```python
from build123d import *

# Parameters (mm, degrees)
MAIN_BLOCK_PROFILE_W            = 44
MAIN_BLOCK_PROFILE_H            = 46
MAIN_BLOCK_PROFILE_R            = 11
MAIN_BLOCK_44MM_DEPTH           = 44
TOP_POCKET_PROFILE_28X28_W      = 28
TOP_POCKET_PROFILE_28X28_H      = 28
TOP_SQUARE_POCKET_28X28X5_DEPTH = 5
SIDE_BOSS_PROFILE_W             = 26
SIDE_BOSS_PROFILE_H             = 30
SIDE_BOSS_PROFILE_W_2           = 14
SIDE_BOSS_PROFILE_H_2           = 16
SIDE_SQUARE_BOSS_23MM_DEPTH     = 23
SIDE_OPENING_PROFILE_W          = 14
SIDE_OPENING_PROFILE_H          = 16
SIDE_OPENING_CUT_DEPTH          = 103.786185842


with BuildPart() as part:
    # Main Block Profile → Main Block 44mm (new body)
    with BuildSketch(Plane.XY):
        Rectangle(MAIN_BLOCK_PROFILE_W, MAIN_BLOCK_PROFILE_H)
        with Locations((0, -1)):
            Circle(MAIN_BLOCK_PROFILE_R, mode=Mode.SUBTRACT)
    extrude(amount=-MAIN_BLOCK_44MM_DEPTH)

    # Top Pocket Profile 28x28 → Top Square Pocket 28x28x5 (cut)
    with BuildSketch(Plane(origin=(0, 23, 0), x_dir=(1, 0, 0), z_dir=(0, 1, 0))):
        with Locations((0, 22)):
            Rectangle(TOP_POCKET_PROFILE_28X28_W, TOP_POCKET_PROFILE_28X28_H)
    extrude(amount=-TOP_SQUARE_POCKET_28X28X5_DEPTH, mode=Mode.SUBTRACT)

    # Side Boss Profile → Side Square Boss 23mm (add)
    with BuildSketch(Plane.ZY.offset(22)):
        with Locations((-16, 0)):
            Rectangle(SIDE_BOSS_PROFILE_W, SIDE_BOSS_PROFILE_H)
        with Locations((-16, 0)):
            Rectangle(SIDE_BOSS_PROFILE_W_2, SIDE_BOSS_PROFILE_H_2, mode=Mode.SUBTRACT)
    side_square_boss_23mm = extrude(amount=SIDE_SQUARE_BOSS_23MM_DEPTH)

    # Side Boss Mirror: Side Square Boss 23mm across plane
    add(side_square_boss_23mm.mirror(Plane(origin=(0, 0, 0), x_dir=(0, 0, 1), z_dir=(1, 0, 0))))

    # Side Opening Profile → Side Opening Cut (cut, through all)
    with BuildSketch(Plane(origin=(45, 0, 0), x_dir=(0, 0, -1), z_dir=(1, 0, 0))):
        with Locations((16, 0)):
            Rectangle(SIDE_OPENING_PROFILE_W, SIDE_OPENING_PROFILE_H)
    extrude(amount=-SIDE_OPENING_CUT_DEPTH, mode=Mode.SUBTRACT)


solid = part.part
```
Work out the finished part from the listing and answer in its coordinate system (mm). A direction names the side the tool comes from. Round coordinates to 2 decimals unless told otherwise and drop trailing zeros. Write each loop counter-clockwise with the first axis right and the second up, starting at its lowest first coordinate (ties: lowest second). Pieces come first, ordered by that corner, then holes. Notation, with made-up numbers: (22, -33.75) - (27, -33.75) arc R24 cw to (27, -14.75) - close; hole circle Ø2 at (67.5, -2). An arc over 180 degrees is marked (long way). Return JSON: item names as keys, results as strings. Group by question number.
Q1. The part is cut by section D-D on y = -1. Write down the section's boundary in (x, z).
Q2. The mould has two halves that part along Y. Classify faces 4 (the flat face through (0, 18, -22)), 5 (the cylindrical face through (5.914, 8.275, -21.692)), 6 (the flat face through (45, 0, -8)): released by +Y, released by -Y, zero draft, split by the parting line, or undercut.
Q3. The part is cut by section C-C on x = -21. Write down the section's boundary in (y, z).
Q4. For faces 1 (the flat face through (26, 0, -9)), 2 (the flat face through (-33, 0, -29)), 3 (the flat face through (33, 0, -3)), determine the directions among +Z, -Z, +X, -X, +Y, -Y from which every point of the face is accessible in a straight line to the end or side of a thin tool.
Q5. Each of these flat-tipped pins is pushed along its axis until it touches: pin 1 Ø8 at (x, y) = (32, -2) entering from +Z; pin 2 Ø18.5 at (x, y) = (-36.5, 1.5) entering from -Z; pin 3 Ø12 at (x, z) = (-29.5, -10) entering from +Y; pin 4 Ø17.5 at (x, y) = (0, -1) entering from -Z. Where does it stop, or does it pass through?
Q6. The part is cut by section B-B on z = -22. Write down the section's boundary in (x, y).
Q7. Find the intervals of material crossed by L1, parallel to Y at x = 0, z = -21; L2, parallel to X at y = -1, z = -25.5; L3, parallel to X at y = -1, z = -34, in increasing order.
Q8. The part is cut by section A-A on x = 0. Write down the section's boundary in (y, z), then the cut area to 3 significant figures.
Solved:
{
 "1": {"outline": "(-45, -29) - (-22, -29) - (-22, -44) - (-11, -44) - (-11, -23) - (-45, -23) - close; (-45, -9) - (-11, -9) - (-11, 0) - (-22, 0) - (-22, -3) - (-45, -3) - close; (11, -44) - (22, -44) - (22, -29) - (45, -29) - (45, -23) - (11, -23) - close; (11, -9) - (45, -9) - (45, -3) - (22, -3) - (22, 0) - (11, 0) - close"},
 "2": {"face 4": "released by +Y", "face 5": "undercut", "face 6": "zero draft"},
 "3": {"outline": "(-23, -44) - (23, -44) - (23, 0) - (-23, 0) - close; hole (-8, -23) - (8, -23) - (8, -9) - (-8, -9) - close"},
 "4": {"face 1": "+X, -X", "face 2": "-Z, -X, +Y, -Y", "face 3": "+Z, +X, +Y, -Y"},
 "5": {"pin 1": "z = -3", "pin 2": "z = -29", "pin 3": "y = 15", "pin 4": "through"},
 "6": {"outline": "(-45, -15) - (-22, -15) - (-22, -23) - (22, -23) - (22, -15) - (45, -15) - (45, -8) - (8.49, -8) arc R11 cw to (-8.49, -8) - (-45, -8) - close; (-45, 8) - (-6.32, 8) arc R11 cw to (6.32, 8) - (45, 8) - (45, 15) - (22, 15) - (22, 23) - (14, 23) - (14, 18) - (-14, 18) - (-14, 23) - (-22, 23) - (-22, 15) - (-45, 15) - close"},
 "7": {"L1": "-23 to -12, 10 to 18", "L2": "-45 to -11, 11 to 45", "L3": "-22 to -11, 11 to 22"},
 "8": {"outline": "(-23, -44) - (-12, -44) - (-12, 0) - (-23, 0) - close; (10, -44) - (23, -44) - (23, -36) - (18, -36) - (18, -8) - (23, -8) - (23, 0) - (10, 0) - close", "area": "916 mm²"}
}
